The model under review builds one solid part; all positions refer to its coordinate system, in mm. A direction names the side the tool comes from. Give positions to 0.01 mm unless a question says otherwise; leave off trailing zeros. Write each loop counter-clockwise with the first axis right and the second up, starting at its lowest first coordinate (ties: lowest second). Pieces come first, ordered by that corner, then holes. Notation, with made-up numbers: (-6, 7.5) - (2, 7.5) arc R31 ccw to (2, 46.5) - close; hole circle Ø3 at (-17.75, 1). An arc over 180 degrees is marked (long way). Write item = value, one per line.
```python
from build123d import *

# Parameters (mm, degrees)
BASE_BLOCK_SKETCH_R   = 28
BASE_BLOCK_SKETCH_R_2 = 16
BASE_BLOCK_DEPTH      = 56
CLAMP_BOSS_DEPTH      = 24
SIDE_WINDOW_CUT_DEPTH = 54
BORE_DEPTH            = 30
CLAMP_SLIT_2_5_DEPTH  = 80


with BuildPart() as part:
    # Base Block Sketch → Base Block (new body)
    with BuildSketch(Plane(origin=(0, 0, 0), x_dir=(0, 0, -1), z_dir=(1, 0, 0))):
        Circle(BASE_BLOCK_SKETCH_R)
        Circle(BASE_BLOCK_SKETCH_R_2, mode=Mode.SUBTRACT)
    extrude(amount=BASE_BLOCK_DEPTH)

    # Clamp Boss Sketch → Clamp Boss (add)
    with BuildSketch(Plane.ZY):
        Polygon((0, 0), (0, 28), (70, 28), (70, -28), (0, -28), align=None)
    extrude(amount=-CLAMP_BOSS_DEPTH)

    # Side Window Sketch → Side Window Cut (cut)
    with BuildSketch(Plane.ZY):
        with BuildLine():
            Line((0, 16), (0, -16))
            ThreePointArc((0, -16), (16, 0), (0, 16))
        make_face()
    extrude(amount=-SIDE_WINDOW_CUT_DEPTH, mode=Mode.SUBTRACT)

    # Bore Sketch → Bore (cut)
    with BuildSketch(Plane.XY.offset(70)):
        with BuildLine():
            Line((24, 16), (24, -16))
            ThreePointArc((24, -16), (8, 0), (24, 16))
        make_face()
    extrude(amount=-BORE_DEPTH, mode=Mode.SUBTRACT)

    # Clamp Slit Sketch → Clamp Slit 2.5 (cut)
    with BuildSketch(Plane(origin=(56, 0, 0), x_dir=(0, 0, -1), z_dir=(1, 0, 0))):
        Polygon((30.140731053, 0), (30.140731053, 2.5), (15.803480629, 2.5), (15.803480629, -2.5), (30.140731053, -2.5), align=None)
    extrude(amount=-CLAMP_SLIT_2_5_DEPTH, mode=Mode.SUBTRACT)


solid = part.part
```
1. Take a section at B-B on z = 8. Give the boundary of the cut face in (x, y), and give its area (3 significant figures).
Findings below:
outline = (0, -28) - (24, -28) - (24, -26.83) - (56, -26.83) - (56, -13.86) - (0, -13.86) - close; (0, 13.86) - (56, 13.86) - (56, 26.83) - (24, 26.83) - (24, 28) - (0, 28) - close
area = 1,510 mm²
2. Take a section at C-C on x = 6.5. Give the boundary of the cut face in (y, z).
Findings below:
outline = (-28, 0) arc R28 ccw to (-2.5, -27.89) - (-2.5, -15.8) arc R16 cw (long way) to (2.5, -15.8) - (2.5, -27.89) arc R28 ccw to (28, 0) - (28, 70) - (-28, 70) - close
3. For line 1 (Y direction, x = 14, z = 0); line 2 (Z direction, x = 39, y = 0); line 3 (Z direction, x = 27, y = 6), list the stretches that pass through material, from the lowest coordinate up. Write a range as from..to.
Findings below:
line_1 = -28..-16, 16..28
line_2 = 16..28
line_3 = -27.35..-14.83, 14.83..27.35
4. Machinability: for faces 1 (the flat face through (24, 0, 35)), 2 (the flat face through (28, 2.5, -22)), 3 (the flat face through (56, -12, -12)), 4 (the cylindrical face through (33.83, 10.54, -25.94)), 5 (the flat face through (0, 0, 33)), which of the approach directions +Z, -Z, +X, -X, +Y, -Y give a long, thin tool a straight path to every point of the face, cutting with its end or side? Answer none if there is none.
Findings below:
face_1 = +Z, +X
face_2 = -Z, +X, -X
face_3 = +Z, -Z, +X, +Y, -Y
face_4 = +X
face_5 = +Z, -Z, -X, +Y, -Y
5. Draft analysis for pull direction Y (two halves, no side actions). For faces 6 (the flat face through (12, 28, 35)), 7 (the flat face through (18, 0, 40)), 8 (the flat face through (12, -28, 35)), state which applies: +Y half, -Y half, draft (parallel to the pull), parting line (faces both ways), or undercut.
Findings below:
face_6 = +Y half
face_7 = undercut
face_8 = -Y half
6. Take a section at D-D on y = 0. Give the boundary of the cut face in (x, z).
Findings below:
outline = (0, 16) - (56, 16) - (56, 28) - (24, 28) - (24, 40) - (8, 40) - (8, 70) - (0, 70) - close
7. Take a section at A-A on y = -10.5. Give the boundary of the cut face in (x, z), and give its area (3 significant figures).
Findings below:
outline = (0, -25.96) - (56, -25.96) - (56, -12.07) - (0, -12.07) - close; (0, 12.07) - (56, 12.07) - (56, 25.96) - (24, 25.96) - (24, 40) - (11.93, 40) - (11.93, 70) - (0, 70) - close
area = 2,250 mm²
8. Insertion check: P1, Ø8, axis at y = 0, z = 35.5, coming from the -X side; P2, Ø6, axis at x = 29, z = -20, coming from the -Y side; P3, Ø6, axis at x = 42.5, y = -10.5, coming from the +Z side; P4, Ø4, axis at x = 32.5, y = -6.5, coming from the +Z side. Each pin has a flat end and moves straight along its axis. Give the tip position at first contact, or say it passes through.
Findings below:
P1 = 0
P2 = -22.25
P3 = 26.98
P4 = 27.64
